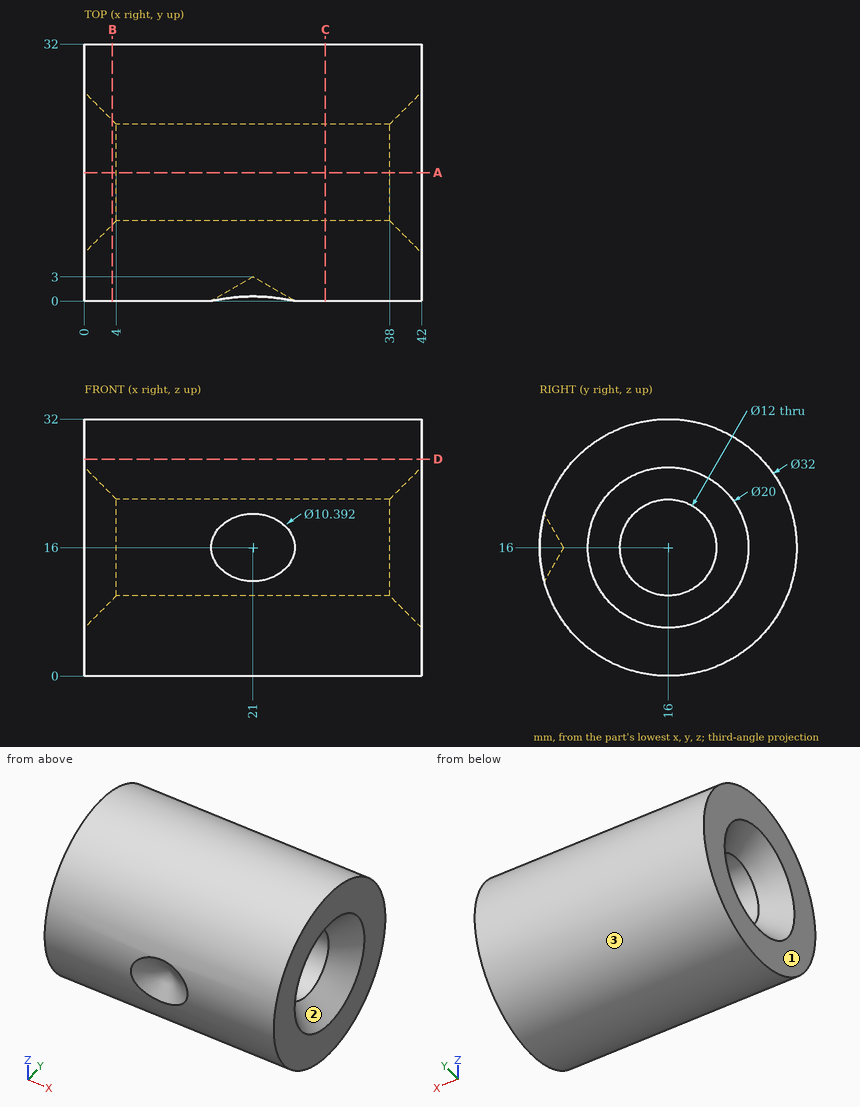
Source: three-view drawing plus pictorial views. Frame: mm from the lowest corner of the part. Give positions to 0.01 mm unless a question says otherwise; leave off trailing zeros. Write each loop counter-clockwise with the first axis right and the second up, starting at its lowest first coordinate (ties: lowest second). Pieces come first, ordered by that corner, then holes. Notation, with made-up numbers: (39, 9.5) -> (81, 9.5) arc R14 ccw to (81, 33.5) -> close; hole circle Ø4 at (-9.5, 64.5). An arc over 180 degrees is marked (long way). Answer in a Markdown table with one row per item.
(1) Section query B-B on x = 3.5. Return loops of the section in (y, z).
Answers below:
| item | result |
|---|---|
| outline | circle Ø32 at (16, 16); hole circle Ø13 at (16, 16) |
(2) Pin query (flat end, axial travel): pin 1 (19 mm diameter, centred on y = 16, z = 16, fed in from -X); pin 2 (8 mm diameter, centred on y = 21, z = 15, fed in from +X); pin 3 (2 mm diameter, centred on y = 23.5, z = 14, fed in from -X). Return the tip coordinate at first contact, or that it passes through.
Answers below:
| item | result |
|---|---|
| pin 1 | x = 0.5 |
| pin 2 | x = 41.1 |
| pin 3 | x = 1.24 |
(3) Ray query, line 1 along Y through (x, z) = (29, 16); line 2 along Y through (x, z) = (20, 12); line 3 along Z through (x, y) = (28, 26). Return the intervals inside material, ascending. Write a range as [from, to].
Answers below:
| item | result |
|---|---|
| line 1 | [0, 10], [22, 32] |
| line 2 | [0.62, 11.53], [20.47, 31.49] |
| line 3 | [3.51, 28.49] |
(4) Section query C-C on x = 30. Return loops of the section in (y, z).
Answers below:
| item | result |
|---|---|
| outline | circle Ø32 at (16, 16); hole circle Ø12 at (16, 16) |
(5) Section query D-D on z = 27. Return loops of the section in (x, y).
Answers below:
| item | result |
|---|---|
| outline | (0, 4.38) -> (42, 4.38) -> (42, 27.62) -> (0, 27.62) -> close |
(6) Draft query along Z for the marked faces 1, 2 and 3. Return one class per face: +Z half, -Z half, draft (parallel to the pull), parting line (faces both ways), or undercut.
Answers below:
| item | result |
|---|---|
| face 1 | draft |
| face 2 | undercut |
| face 3 | parting line |
(7) Section query A-A on y = 16. Return loops of the section in (x, z), then the cut area to 3 significant figures.
Answers below:
| item | result |
|---|---|
| outline | (0, 0) -> (42, 0) -> (42, 6) -> (38, 10) -> (4, 10) -> (0, 6) -> close; (0, 26) -> (4, 22) -> (38, 22) -> (42, 26) -> (42, 32) -> (0, 32) -> close |
| area | 808 mm^2 |
